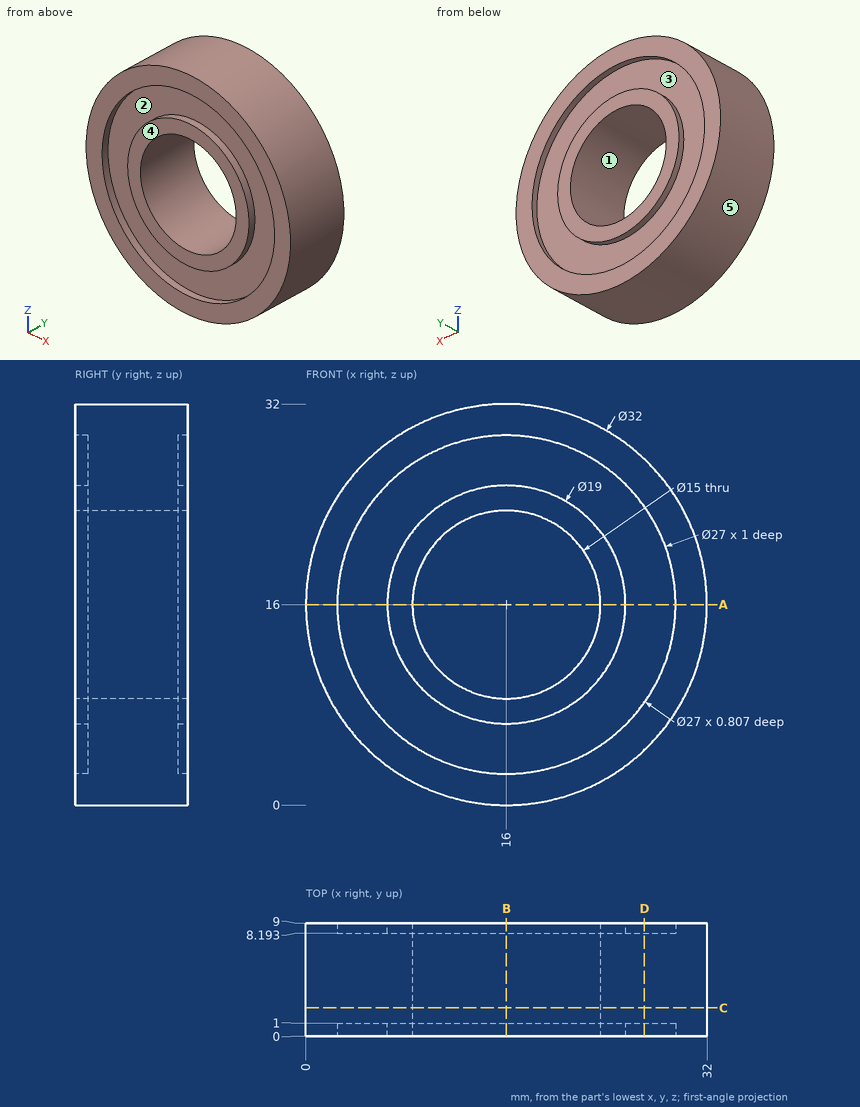
Drawing for the job (mm, zero at the part's lowest x, y, z). A direction names the side the tool comes from. Coordinates: 2 decimals unless noted, no trailing zeros. Order: outer loops, then holes, each group sorted by start corner. A loop starts at its lowest first (then second) coordinate and runs counter-clockwise, first axis right, second up. Notation, with made-up numbers: (6, 49) -> (16, 49) arc R21 cw to (16, 79) -> close; hole circle Ø1 at (76.5, 39.25). An arc over 180 degrees is marked (long way). Answer in a Markdown table with one row per item.
1) Band-saw the part on B-B (x = 16). List the corners of the cut face in (y, z).
Check values:
| item | result |
|---|---|
| outline | (0, 0) -> (9, 0) -> (9, 2.5) -> (8.19, 2.5) -> (8.19, 6.5) -> (9, 6.5) -> (9, 8.5) -> (0, 8.5) -> (0, 6.5) -> (1, 6.5) -> (1, 2.5) -> (0, 2.5) -> close; (0, 23.5) -> (9, 23.5) -> (9, 25.5) -> (8.19, 25.5) -> (8.19, 29.5) -> (9, 29.5) -> (9, 32) -> (0, 32) -> (0, 29.5) -> (1, 29.5) -> (1, 25.5) -> (0, 25.5) -> close |
2) Band-saw the part on A-A (z = 16). List the corners of the cut face in (x, y), and give its area (3 significant figures).
Check values:
| item | result |
|---|---|
| outline | (0, 0) -> (2.5, 0) -> (2.5, 1) -> (6.5, 1) -> (6.5, 0) -> (8.5, 0) -> (8.5, 9) -> (6.5, 9) -> (6.5, 8.19) -> (2.5, 8.19) -> (2.5, 9) -> (0, 9) -> close; (23.5, 0) -> (25.5, 0) -> (25.5, 1) -> (29.5, 1) -> (29.5, 0) -> (32, 0) -> (32, 9) -> (29.5, 9) -> (29.5, 8.19) -> (25.5, 8.19) -> (25.5, 9) -> (23.5, 9) -> close |
| area | 139 mm2 |
3) Flat gauge pins, fed straight in: P1, Ø2, axis at x = 4, y = 2, coming from the -Z side; P2, Ø1.5, axis at y = 8, z = 17, coming from the +X side; P3, Ø3, axis at x = 27.5, y = 5, coming from the +Z side. Where does each tip first touch, or does it go through?
Check values:
| item | result |
|---|---|
| P1 | z = 4.38 |
| P2 | x = 32 |
| P3 | z = 28.49 |
4) Mould opens along Z. For the marked faces 3, 4 and 5 say: pulls with the +Z half, pulls with the -Z half, needs draft (parallel to the pull), parting line crosses it, or undercut.
Check values:
| item | result |
|---|---|
| face 3 | undercut |
| face 4 | needs draft |
| face 5 | parting line crosses it |
5) Drill centre lines: line 1 (Z direction, x = 16, y = 0.6); line 2 (Z direction, x = 19, y = 8.75). Where is each one in solid material? Low to high.
Check values:
| item | result |
|---|---|
| line 1 | 0 to 2.5, 6.5 to 8.5, 23.5 to 25.5, 29.5 to 32 |
| line 2 | 0.28 to 2.84, 6.99 to 9.13, 22.87 to 25.01, 29.16 to 31.72 |
6) Band-saw the part on C-C (y = 2.25). List the corners of the cut face in (x, z).
Check values:
| item | result |
|---|---|
| outline | circle Ø32 at (16, 16); hole circle Ø15 at (16, 16) |
7) Which spindle directions (+Z, -Z, +X, -X, +Y, -Y) get a long thin tool onto all of the face, cutting with end or side? Do the marked faces 1 and 2. Say none if no direction does.
Check values:
| item | result |
|---|---|
| face 1 | +Y, -Y |
| face 2 | -Y |
8) Band-saw the part on D-D (x = 27). List the corners of the cut face in (y, z).
Check values:
| item | result |
|---|---|
| outline | (0, 4.38) -> (9, 4.38) -> (9, 8.17) -> (8.19, 8.17) -> (8.19, 23.83) -> (9, 23.83) -> (9, 27.62) -> (0, 27.62) -> (0, 23.83) -> (1, 23.83) -> (1, 8.17) -> (0, 8.17) -> close |
